Here's how the part is built. I have some questions about the finished solid (model axes, mm). Round coordinates to 2 decimals unless told otherwise and drop trailing zeros. Write each loop counter-clockwise with the first axis right and the second up, starting at its lowest first coordinate (ties: lowest second). Pieces come first, ordered by that corner, then holes. Notation, with made-up numbers: M 67,20 L 93,20 A31 cw 93,51 Z; hole C 45.25,78.5 d4. An arc over 180 degrees is marked long. Write item = value, one per line. Start each with the question number.
(1) I want a section at C-C (y = 0.3). List the corners of the cut face in (x, z) for me, and give its area (3 significant figures).
(2) I want a section at A-A (x = -5). List the corners of the cut face in (y, z) for me, and give its area (3 significant figures).
(3) I want a section at B-B (z = 0.15). List the corners of the cut face in (x, y) for me, and give its area (3 significant figures).
(4) If we mould it in two halves opening along Y, with no side actions, what happens to faces 1 (the cylindrical face through (-4.49, -0.21, -0.01)), 2 (the flat face through (0, 1, 0)), 3 (the flat face through (0, -1, 0))? For each: released by +Y, released by -Y, zero draft, split by the parting line, or undercut.
(5) I need wall thicknesses on line 1 along X through (y, z) = (0.05, 0.2); line 2 along Y through (x, z) = (-10, -0.3); line 3 along X through (y, z) = (0.8, -0.35). Which ranges of each line are inside material? Lowest first, please.
(6) Will this pin go through, and if not, where does the flat tip stop? pin 1 Ø0.9 at (x, y) = (-5, 0) entering from -Z.
```python
from build123d import *

# Parameters (mm, degrees)
SKETCH1_R           = 0.55
THIGH1_LENGTH_DEPTH = 0.5


with BuildPart() as part:
    # Sketch1 → Thigh1 length (new, symmetric)
    with BuildSketch(Plane.XY):
        with BuildLine():
            Line((-10, 1), (10, 1))
            ThreePointArc((10, 1), (11, 0), (10, -1))
            Line((10, -1), (-10, -1))
            ThreePointArc((-10, -1), (-11, 0), (-10, 1))
        make_face()
        with Locations((-10, 0)):
            Circle(SKETCH1_R, mode=Mode.SUBTRACT)
        with Locations((10, 0)):
            Circle(SKETCH1_R, mode=Mode.SUBTRACT)
        with Locations((-5, 0)):
            Circle(SKETCH1_R, mode=Mode.SUBTRACT)
    extrude(amount=THIGH1_LENGTH_DEPTH, both=True)


solid = part.part
```
Returned:
q1.outline = M -10.95,-0.5 L -10.46,-0.5 L -10.46,0.5 L -10.95,0.5 Z; M -9.54,-0.5 L -5.46,-0.5 L -5.46,0.5 L -9.54,0.5 Z; M -4.54,-0.5 L 9.54,-0.5 L 9.54,0.5 L -4.54,0.5 Z; M 10.46,-0.5 L 10.95,-0.5 L 10.95,0.5 L 10.46,0.5 Z
q1.area = 19.1 mm²
q2.outline = M -1,-0.5 L -0.55,-0.5 L -0.55,0.5 L -1,0.5 Z; M 0.55,-0.5 L 1,-0.5 L 1,0.5 L 0.55,0.5 Z
q2.area = 0.900 mm²
q3.outline = M -10,-1 L 10,-1 A1 ccw 10,1 L -10,1 A1 ccw Z; hole C -10,0 d1.1; hole C -5,0 d1.1; hole C 10,0 d1.1
q3.area = 40.3 mm²
q4.face_1 = undercut
q4.face_2 = released by +Y
q4.face_3 = released by -Y
q5.line_1 = -11 to -10.55, -9.45 to -5.55, -4.45 to 9.45, 10.55 to 11
q5.line_2 = -1 to -0.55, 0.55 to 1
q5.line_3 = -10.6 to 10.6
q6.pin_1 = through
